CAD build for the part. Positions are in the model's coordinates, mm. A direction names the side the tool comes from. Round coordinates to 2 decimals unless told otherwise and drop trailing zeros. Loops run counter-clockwise (first coordinate to the right, second up) from the corner with the lowest first, then second, coordinate; pieces in that order, holes last.
```python
from build123d import *

# Parameters (mm, degrees)
SKETCH_1_W      = 30
SKETCH_1_H      = 60
EXTRUDE_1_DEPTH = 374
SHELL_1_T       = -2


with BuildPart() as part:
    # 草图1 → 凸台-拉伸1 (new, symmetric)
    with BuildSketch(Plane.XY):
        Rectangle(SKETCH_1_W, SKETCH_1_H)
    extrude(amount=EXTRUDE_1_DEPTH, both=True)

    # 抽壳1
    shell_1_openings = [part.faces().sort_by_distance(p)[0] for p in [
        (0, 0, 374),
        (0, 0, -374),
        (0, 30, 0),
    ]]
    offset(amount=SHELL_1_T, openings=shell_1_openings, kind=Kind.INTERSECTION)


solid = part.part
```
Item 1: Probe line 1 (X direction, y = -25.5, z = -251); line 2 (Y direction, x = -3.25, z = 183). List the from-to ranges inside material, lowest first.
Answers follow:
line 1: x = -15 to -13, 13 to 15
line 2: y = -30 to -28
Item 2: Cut at B-B, the plane z = 1. Give the cut face in (x, y), plus the area to 3 significant figures.
Answers follow:
outline: (-15, -30) - (15, -30) - (15, 30) - (13, 30) - (13, -28) - (-13, -28) - (-13, 30) - (-15, 30) - close
area: 292 mm2
Item 3: Flat gauge pin, fed straight in: P1, Ø10, axis at x = 3.5, z = -36.5, coming from the +Y side. Where does the tip first touch, or does it go through?
Answers follow:
P1: stops at y = -28
Item 4: 3-axis set-ups, long thin cutter, end or side, ignore diameter. For faces 4 (the flat face through (-13.4, -6.5, -374)), 5 (the flat face through (-13, 1, 5)): which of +Z, -Z, +X, -X, +Y, -Y reach the whole face in a straight line?
Answers follow:
face 4: -Z, +X, -X, +Y, -Y
face 5: +Z, -Z, +Y
Item 5: Cut at A-A, the plane y = -6. Give the cut face in (x, z), plus the area to 3 significant figures.
Answers follow:
outline: (-15, -374) - (-13, -374) - (-13, 374) - (-15, 374) - close; (13, -374) - (15, -374) - (15, 374) - (13, 374) - close
area: 2,990 mm2
Item 6: Cut at C-C, the plane x = 5.5. Give the cut face in (y, z), plus the area to 3 significant figures.
Answers follow:
outline: (-30, -374) - (-28, -374) - (-28, 374) - (-30, 374) - close
area: 1,500 mm2
Item 7: Two-plate mould, pull along Y, no slides. Class faces 1 (the flat face through (0, -28, 5)), 2 (the flat face through (-13.4, -6.5, 374)), 3 (the flat face through (0, -30, 5)): released by +Y, released by -Y, zero draft, split by the parting line, or undercut.
Answers follow:
face 1: released by +Y
face 2: zero draft
face 3: released by -Y
